Geometry: final body of the model. Coordinates: model frame, mm. Give positions to 0.01 mm unless a question says otherwise; leave off trailing zeros. Loops run counter-clockwise (first coordinate to the right, second up) from the corner with the lowest first, then second, coordinate; pieces in that order, holes last. Notation, with made-up numbers: (87, 73) - (109, 73) arc R12 ccw to (109, 90) - close; hole circle Ø9 at (78.25, 62.25). An arc over 180 degrees is marked (long way). Use CSV: the item, a comma, the result in double quotes. Start each with the question number.
```python
from build123d import *

# Parameters (mm, degrees)
SKETCH_1_W             = 200
SKETCH_1_H             = 90
EXTRUDE_1_DEPTH        = 10
HOLE_WIZARD_M6_1_D     = 5
HOLE_WIZARD_M8_1_D     = 10
HOLE_WIZARD_M8_1_DEPTH = 30
HOLE_WIZARD_M8_1_TIP   = 3.004303095


with BuildPart() as part:
    # 草图1 → 凸台-拉伸1 (new body)
    with BuildSketch(Plane.XY):
        Rectangle(SKETCH_1_W, SKETCH_1_H)
    extrude(amount=EXTRUDE_1_DEPTH)

    # M6 螺纹孔1 (through all)
    with Locations(Plane(origin=(0, 0, 0), x_dir=(-1, 0, 0), z_dir=(0, 0, -1))):
        with Locations((85, 30), (35, -30), (85, -30), (35, 30)):
            Hole(HOLE_WIZARD_M6_1_D / 2)

    # M8 间隙孔1
    with Locations(Plane.XY.offset(10)):
        with Locations((85, -30), (85, 30), (25, -30), (25, 30)):
            Hole(HOLE_WIZARD_M8_1_D / 2, depth=HOLE_WIZARD_M8_1_DEPTH)
            with Locations((0, 0, -(HOLE_WIZARD_M8_1_DEPTH + HOLE_WIZARD_M8_1_TIP / 2))):  # 118° drill point
                Cone(0, HOLE_WIZARD_M8_1_D / 2, HOLE_WIZARD_M8_1_TIP, mode=Mode.SUBTRACT)


solid = part.part
```
Item 1: Pin query (flat end, axial travel): pin 1 Ø9 at (x, y) = (25, -30) entering from -Z. Return the tip coordinate at first contact, or that it passes through.
Item 2: Ray query, probe 1 along Y at (x, z) = (25, 5.25); probe 2 along Y at (x, z) = (-35, 6); probe 3 along X at (y, z) = (31, 2.75). Return the intervals inside material, ascending.
Item 3: Mould query, pull axis Y, two halves, no side actions, for faces 1 (the cylindrical face through (-33.66, 32.11, 5.07)), 2 (the cylindrical face through (30, -30, 5)), 3 (the flat face through (-1, 1, 10)), 4 (the flat face through (-1, -45, 5)). Classes: pulls with the +Y half, pulls with the -Y half, needs draft (parallel to the pull), parting line crosses it, or undercut.
Item 4: Section D-D (x = 25). Output: boundary loops of the cut face in (y, z), plus the area to 3 significant figures.
Item 5: Section B-B (y = -30). Output: boundary loops of the cut face in (x, z).
Item 6: Section A-A (x = -35). Output: boundary loops of the cut face in (y, z).
Item 7: Section C-C (z = 5.75). Give the number of separate pieces and of enclosed holes in the cut face, plus the area to 3 significant figures.
Outcome:
1,pin 1,"passes through"
2,probe 1,"y = -45 to -35, -25 to 25, 35 to 45"
2,probe 2,"y = -45 to -32.5, -27.5 to 27.5, 32.5 to 45"
2,probe 3,"x = -100 to -87.29, -82.71 to -37.29, -32.71 to 20.1, 29.9 to 80.1, 89.9 to 100"
3,face 1,"undercut"
3,face 2,"undercut"
3,face 3,"needs draft"
3,face 4,"pulls with the -Y half"
4,outline,"(-45, 0) - (-35, 0) - (-35, 10) - (-45, 10) - close; (-25, 0) - (25, 0) - (25, 10) - (-25, 10) - close; (35, 0) - (45, 0) - (45, 10) - (35, 10) - close"
4,area,"700 mm2"
5,outline,"(-100, 0) - (-87.5, 0) - (-87.5, 10) - (-100, 10) - close; (-82.5, 0) - (-37.5, 0) - (-37.5, 10) - (-82.5, 10) - close; (-32.5, 0) - (20, 0) - (20, 10) - (-32.5, 10) - close; (30, 0) - (80, 0) - (80, 10) - (30, 10) - close; (90, 0) - (100, 0) - (100, 10) - (90, 10) - close"
6,outline,"(-45, 0) - (-32.5, 0) - (-32.5, 10) - (-45, 10) - close; (-27.5, 0) - (27.5, 0) - (27.5, 10) - (-27.5, 10) - close; (32.5, 0) - (45, 0) - (45, 10) - (32.5, 10) - close"
7,separate pieces,"1"
7,enclosed holes,"8"
7,area,"17,600 mm2"
